Read the model definition and answer for the solid it produces. Units are mm, in the model's axes. Face numbers are marked on the shaded views. Coordinates: 2 decimals unless noted, no trailing zeros. Loops run counter-clockwise (first coordinate to the right, second up) from the corner with the lowest first, then second, coordinate; pieces in that order, holes last.
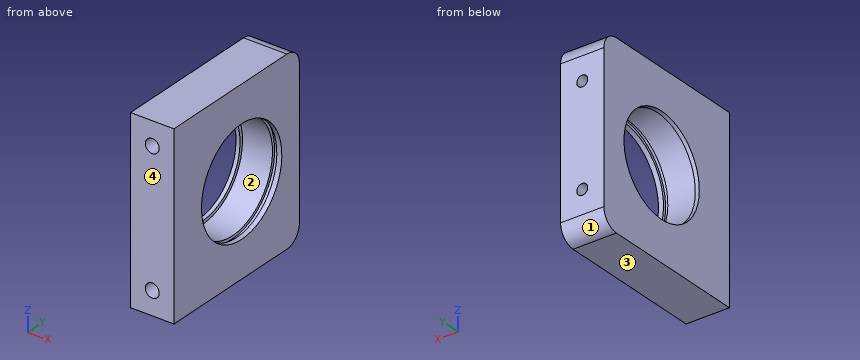
from build123d import *

# Parameters (mm, degrees)
EXTRUDE_1_DEPTH        = 27
SKETCH_2_R             = 16
CUT_EXTRUDE_1_DEPTH    = 107.437775249
EXTRUDE_START          = -1.2
SKETCH_3_R             = 16
SKETCH_3_R_2           = 15
EXTRUDE_1_2_DEPTH      = 1.2
SKETCH_4_W             = 1.3
SKETCH_4_H             = 0.85
SKETCH_5_W             = 103
SKETCH_5_H             = 105
EXTRUDE_2_DEPTH        = 13
FILLET_1_R             = 5
CUT_EXTRUDE_2_DEPTH    = 13
HOLE_WIZARD_M5_1_D     = 4.2
HOLE_WIZARD_M5_1_DEPTH = 12.4
HOLE_WIZARD_M5_1_TIP   = 1.2618073
HOLE_WIZARD_M4_1_D     = 3.3
HOLE_WIZARD_M4_1_DEPTH = 10.1
HOLE_WIZARD_M4_1_TIP   = 0.991420021


with BuildPart() as part:
    # 草图1 → Extrude 1 (new, symmetric)
    with BuildSketch(Plane.XY):
        Polygon((90, 0), (0, 0), (0, 50), (-13, 50), (-13, -13), (90, -13), align=None)
    extrude(amount=EXTRUDE_1_DEPTH, both=True)

    # 草图2 → 切除-拉伸1 (cut, through all)
    with BuildSketch(Plane(origin=(0, 0, 0), x_dir=(0, 0, -1), z_dir=(1, 0, 0))):
        with Locations((0, 27)):
            Circle(SKETCH_2_R)
    extrude(amount=-CUT_EXTRUDE_1_DEPTH, mode=Mode.SUBTRACT)

    # 草图3 → Extrude 1 2 (add)
    with BuildSketch(Plane.ZY.offset(13).offset(EXTRUDE_START)):
        with Locations(Location((0, 27, 0), (0, 0, 180))):
            Circle(SKETCH_3_R)
        with Locations((0, 27)):
            Circle(SKETCH_3_R_2, mode=Mode.SUBTRACT)
    extrude(amount=EXTRUDE_1_2_DEPTH)

    # 草图4 → 切除-旋转1 (revolve, cut)
    with BuildSketch(Plane.XY, mode=Mode.PRIVATE) as cut_revolve_1_sk:
        with Locations((-2.15, 43.425)):
            Rectangle(SKETCH_4_W, SKETCH_4_H)
    revolve(cut_revolve_1_sk.sketch.rotate(Axis((-11.8, 27, 0), (1, 0, 0)), 90), axis=Axis((-11.8, 27, 0), (1, 0, 0)), mode=Mode.SUBTRACT)

    # 草图5 → 凸台-拉伸2 (add)
    with BuildSketch(Plane(origin=(0, 0, 0), x_dir=(1, 0, 0), z_dir=(0, 1, 0))):
        with Locations((38.5, 0)):
            Rectangle(SKETCH_5_W, SKETCH_5_H)
    extrude(amount=-EXTRUDE_2_DEPTH)

    # 圆角1
    fillet_1_edges = [part.edges().sort_by_distance(p)[0] for p in [
        (-6.5, 50, 27),
        (-13, -6.5, 52.5),
        (90, -6.5, -52.5),
        (90, -6.5, 52.5),
        (-13, -6.5, -52.5),
        (-6.5, 50, -27),
    ]]
    fillet(fillet_1_edges, radius=FILLET_1_R)

    # 草图6 → 切除-拉伸2 (cut)
    with BuildSketch(Plane.XZ.offset(13)):
        with BuildLine():
            Line((-13, 47.5), (-13, -47.5))
            ThreePointArc((-13, -47.5), (-11.535533906, -51.035533906), (-8, -52.5))
            Line((-8, -52.5), (85, -52.5))
            ThreePointArc((85, -52.5), (88.535533906, -51.035533906), (90, -47.5))
            Line((90, -47.5), (90, 47.5))
            ThreePointArc((90, 47.5), (88.535533906, 51.035533906), (85, 52.5))
            Line((85, 52.5), (-8, 52.5))
            ThreePointArc((-8, 52.5), (-11.535533906, 51.035533906), (-13, 47.5))
        make_face()
    extrude(amount=-CUT_EXTRUDE_2_DEPTH, mode=Mode.SUBTRACT)

    # M5 螺纹孔1
    with Locations(Plane(origin=(-6.5, 0, 20), x_dir=(0, 0, -1), z_dir=(0, -1, 0))):
        with Locations((0, 0), (40, 0)):
            Hole(HOLE_WIZARD_M5_1_D / 2, depth=HOLE_WIZARD_M5_1_DEPTH)
            with Locations((0, 0, -(HOLE_WIZARD_M5_1_DEPTH + HOLE_WIZARD_M5_1_TIP / 2))):  # 118° drill point
                Cone(0, HOLE_WIZARD_M5_1_D / 2, HOLE_WIZARD_M5_1_TIP, mode=Mode.SUBTRACT)

    # M4 螺纹孔1
    with Locations(Plane(origin=(-6.5, 50, -15), x_dir=(1, 0, 0), z_dir=(0, 1, 0))):
        with Locations((0, 0), (0, -30)):
            Hole(HOLE_WIZARD_M4_1_D / 2, depth=HOLE_WIZARD_M4_1_DEPTH)
            with Locations((0, 0, -(HOLE_WIZARD_M4_1_DEPTH + HOLE_WIZARD_M4_1_TIP / 2))):  # 118° drill point
                Cone(0, HOLE_WIZARD_M4_1_D / 2, HOLE_WIZARD_M4_1_TIP, mode=Mode.SUBTRACT)


solid = part.part
Item 1: A cutting plane is placed at D-D on y = 27. Determine the outline of the cut face in (x, z), then the cut area to 3 significant figures.
Numbers:
outline: (-13, -27) - (0, -27) - (0, -16) - (-1.5, -16) - (-1.5, -16.85) - (-2.8, -16.85) - (-2.8, -16) - (-11.8, -16) - (-11.8, -15) - (-13, -15) - close; (-13, 15) - (-11.8, 15) - (-11.8, 16) - (-2.8, 16) - (-2.8, 16.85) - (-1.5, 16.85) - (-1.5, 16) - (0, 16) - (0, 27) - (-13, 27) - close
area: 286 mm2
Item 2: Determine the mould class of the marked faces 1, 2, 3 and 4 for opening direction Y: released by +Y, released by -Y, zero draft, split by the parting line, or undercut.
Numbers:
face 1: released by +Y
face 2: undercut
face 3: zero draft
face 4: released by -Y
Item 3: A cutting plane is placed at B-B on z = 0. Determine the outline of the cut face in (x, y), then the cut area to 3 significant figures.
Numbers:
outline: (-13, 0) - (0, 0) - (0, 11) - (-1.5, 11) - (-1.5, 10.15) - (-2.8, 10.15) - (-2.8, 11) - (-11.8, 11) - (-11.8, 12) - (-13, 12) - close; (-13, 42) - (-11.8, 42) - (-11.8, 43) - (-2.8, 43) - (-2.8, 43.85) - (-1.5, 43.85) - (-1.5, 43) - (0, 43) - (0, 50) - (-13, 50) - close
area: 234 mm2
Item 4: Find the intervals of material crossed by line 1 along Z through (x, y) = (-6.5, 44.5); line 2 along Y through (x, z) = (-12.05, 0); line 3 along Z through (x, y) = (-0.55, 27), in increasing order.
Numbers:
line 1: z = -27 to -16.65, -13.35 to 13.35, 16.65 to 27
line 2: y = 0 to 12, 42 to 50
line 3: z = -27 to -16, 16 to 27
Item 5: Given pin 1 (1 mm diameter, centred on y = 41.5, z = 1.5, fed in from +X), flat-ended and moving along its own axis, determine where the tip first touches the part or whether it passes through.
Numbers:
pin 1: stops at x = -11.8
Item 6: A cutting plane is placed at C-C on x = -10. Determine the outline of the cut face in (y, z).
Numbers:
outline: (0, -27) - (45, -27) arc R5 ccw to (50, -22) - (50, 22) arc R5 ccw to (45, 27) - (0, 27) - close; hole circle Ø32 at (27, 0)
Item 7: A cutting plane is placed at A-A on y = 41. Determine the outline of the cut face in (x, z).
Numbers:
outline: (-13, -27) - (0, -27) - (0, -7.75) - (-1.5, -7.75) - (-1.5, -9.38) - (-2.8, -9.38) - (-2.8, -7.75) - (-11.8, -7.75) - (-11.8, -5.39) - (-13, -5.39) - close; (-13, 5.39) - (-11.8, 5.39) - (-11.8, 7.75) - (-2.8, 7.75) - (-2.8, 9.38) - (-1.5, 9.38) - (-1.5, 7.75) - (0, 7.75) - (0, 27) - (-13, 27) - close; hole circle Ø3.3 at (-6.5, -15); hole circle Ø3.3 at (-6.5, 15)
